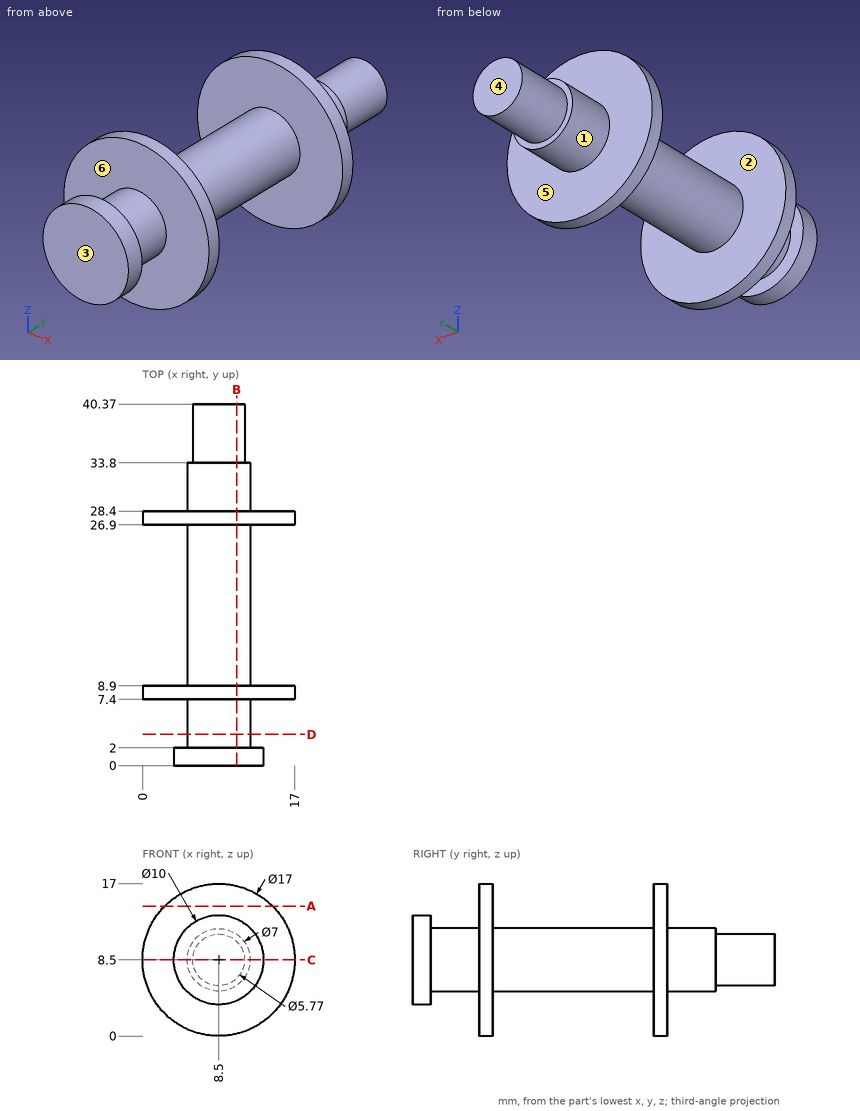
The figure shows three views and two pictorial views of one solid part (mm, origin at its lowest corner). Answer the questions. A direction names the side the tool comes from. Give positions to 0.01 mm unless a question says otherwise; leave off trailing zeros. Loops run counter-clockwise (first coordinate to the right, second up) from the corner with the lowest first, then second, coordinate; pieces in that order, holes last. Notation, with made-up numbers: (17.25, 71) -> (53.25, 71) arc R15 cw to (53.25, 97) -> close; hole circle Ø3 at (7, 85.25). An arc over 180 degrees is marked (long way). Use CSV: the item, a comma, the result in double quotes.
1. The part is cut by section D-D (y = 3.5). Write down the section's boundary in (x, z).
Found:
outline,"circle Ø7 at (8.5, 8.5)"
2. The mould has two halves that part along Y. Classify the marked faces 1, 2, 3 and 4: +Y half, -Y half, draft (parallel to the pull), parting line (faces both ways), or undercut.
Found:
face 1,"draft"
face 2,"undercut"
face 3,"-Y half"
face 4,"+Y half"
3. Flat-ended cylindrical pins translate along their axes: pin 1 Ø1.5 at (y, z) = (21, 9) entering from +X; pin 2 Ø8 at (y, z) = (8, 14.5) entering from -X; pin 3 Ø4 at (x, y) = (11, 10.5) entering from +Z. Find the tip coordinate at first contact, or state that the pin passes through.
Found:
pin 1,"x = 12"
pin 2,"x = 0.24"
pin 3,"z = 16.9"
4. The part is cut by section B-B (x = 10.5). Write down the section's boundary in (y, z).
Found:
outline,"(0, 3.92) -> (2, 3.92) -> (2, 5.63) -> (7.4, 5.63) -> (7.4, 0.24) -> (8.9, 0.24) -> (8.9, 5.63) -> (26.9, 5.63) -> (26.9, 0.24) -> (28.4, 0.24) -> (28.4, 5.63) -> (33.8, 5.63) -> (33.8, 6.42) -> (40.37, 6.42) -> (40.37, 10.58) -> (33.8, 10.58) -> (33.8, 11.37) -> (28.4, 11.37) -> (28.4, 16.76) -> (26.9, 16.76) -> (26.9, 11.37) -> (8.9, 11.37) -> (8.9, 16.76) -> (7.4, 16.76) -> (7.4, 11.37) -> (2, 11.37) -> (2, 13.08) -> (0, 13.08) -> close"
5. The part is cut by section C-C (z = 8.5). Write down the section's boundary in (x, y) (3 decimals), then the cut area to 3 significant figures.
Found:
outline,"(0, 7.4) -> (5, 7.4) -> (5, 2) -> (3.5, 2) -> (3.5, 0) -> (13.5, 0) -> (13.5, 2) -> (12, 2) -> (12, 7.4) -> (17, 7.4) -> (17, 8.9) -> (12, 8.9) -> (12, 26.9) -> (17, 26.9) -> (17, 28.4) -> (12, 28.4) -> (12, 33.8) -> (11.385, 33.8) -> (11.385, 40.37) -> (5.615, 40.37) -> (5.615, 33.8) -> (5, 33.8) -> (5, 28.4) -> (0, 28.4) -> (0, 26.9) -> (5, 26.9) -> (5, 8.9) -> (0, 8.9) -> close"
area,"311 mm^2"
6. The part is cut by section A-A (z = 14.5). Write down the section's boundary in (x, y), then the cut area to 3 significant figures.
Found:
outline,"(2.48, 7.4) -> (14.52, 7.4) -> (14.52, 8.9) -> (2.48, 8.9) -> close; (2.48, 26.9) -> (14.52, 26.9) -> (14.52, 28.4) -> (2.48, 28.4) -> close"
area,"36.1 mm^2"
7. A tool of negligible diameter and unlimited length cuts with its end or side. For the marked faces 5 and 6, from which of +Z, -Z, +X, -X, +Y, -Y can it reach the whole face along a straight path? Write none if from no direction.
Found:
face 5,"+Y"
face 6,"none"
8. Straight lines are drawn through the part: line 1 (Y direction, x = 8.25, z = 12.75); line 2 (Y direction, x = 15.5, z = 4); line 3 (Y direction, x = 11.5, z = 9). For each, find the intervals that lie inside material, in ascending order.
Found:
line 1,"0 to 2, 7.4 to 8.9, 26.9 to 28.4"
line 2,"7.4 to 8.9, 26.9 to 28.4"
line 3,"0 to 33.8"
